Source: CAD feature listing. Evaluate the final solid. Frame: model axes, mm. A direction names the side the tool comes from. Give positions to 0.01 mm unless a question says otherwise; leave off trailing zeros. Order: outer loops, then holes, each group sorted by start corner. A loop starts at its lowest first (then second) coordinate and runs counter-clockwise, first axis right, second up. Notation, with made-up numbers: M 6.5,4 L 10.5,4 A16 ccw 10.5,16 Z; hole C 47.5,83 d2. An arc over 180 degrees is marked long. Answer as a JSON object with one key per item and string values. Group by question number.
1. Set-up query: faces 1 (the flat face through (15, 30, 15)), 2 (the flat face through (22.5, 55, 15)), 3 (the flat face through (65, 25, 15)), 4 (the cylindrical face through (3.7, 10.5, 13)). Return all of +Z, -Z, +X, -X, +Y, -Y with unobstructed straight access to the full face (end or side cutting, diameter ignored); none if empty.
2. Section query D-D (x = 25). Output: boundary loops of the cut face in (y, z), plus the area to 3 significant figures.
3. Section query B-B (y = 58). Output: boundary loops of the cut face in (x, z).
4. Material intervals for L1, parallel to Y at x = 6.25, z = 15; L2, parallel to Z at x = 2.5, y = 58; L3, parallel to X at y = 41.5, z = 13, sorted ascending. Write a range as [from, to].
5. Section query A-A (y = 12). Output: boundary loops of the cut face in (x, z), plus the area to 3 significant figures.
6. Pin query (flat end, axial travel): P1, Ø5, axis at x = 59, z = 26, coming from the +Y side; P2, Ø6, axis at x = 30.5, z = 17, coming from the -Y side; P3, Ø8, axis at y = 39.5, z = 7.5, coming from the +X side; P4, Ø7.5, axis at x = 13, z = 19, coming from the +Y side. Return the tip coordinate at first contact, or that it passes through.
7. Section query C-C (z = 15). Count the separate pieces of the cut face and the enclosed holes in it, plus the area to 3 significant figures.
8. Pull-direction query (X, two-part tool) for faces 5 (the flat face through (7.5, 15, 15)), 6 (the cylindrical face through (4, 68, 29)), 7 (the flat face through (15, 40, 15)), 8 (the flat face through (30, 50, 15)); classes: +X half, -X half, draft (parallel to the pull), parting line (faces both ways), or undercut.
from build123d import *

# Parameters (mm, degrees)
BOSS_EXTRUDE1_DEPTH = 30
SKETCH4_R           = 9
CUT_EXTRUDE2_DEPTH  = 25
SKETCH5_W           = 15
SKETCH5_H           = 30
CUT_EXTRUDE3_DEPTH  = 111.453610172
SKETCH6_R           = 2.5
CUT_EXTRUDE4_DEPTH  = 25
FILLET1_R           = 5
FILLET2_R           = 10


with BuildPart() as part:
    # Sketch1 → Boss-Extrude1 (new body)
    with BuildSketch(Plane.XY):
        Polygon((0, 0), (0, 70), (30, 70), (30, 30), (80, 30), (80, 0), align=None)
    extrude(amount=BOSS_EXTRUDE1_DEPTH)

    # Sketch4 → Cut-Extrude2 (cut)
    with BuildSketch(Plane(origin=(0, 0, 0), x_dir=(-1, 0, 0), z_dir=(0, -1, 0))):
        with Locations(Location((-65, -15, 0), (0, 0, 180))):
            Circle(SKETCH4_R)
    extrude(amount=-CUT_EXTRUDE2_DEPTH, mode=Mode.SUBTRACT)

    # Sketch5 → Cut-Extrude3 (cut, through all)
    with BuildSketch(Plane(origin=(0, 0, 0), x_dir=(-1, 0, 0), z_dir=(0, 0, -1))):
        with Locations((-15, 55)):
            Rectangle(SKETCH5_W, SKETCH5_H)
        with Locations((-15, 15)):
            Rectangle(SKETCH5_W, SKETCH5_H)
    extrude(amount=-CUT_EXTRUDE3_DEPTH, mode=Mode.SUBTRACT)

    # Sketch6 → Cut-Extrude4 (cut, symmetric)
    with BuildSketch(Plane.ZY.offset(-22.5)):
        with Locations(Location((15, 58, 0), (0, 0, 270))):
            Circle(SKETCH6_R)
        with Locations((15, 12)):
            Circle(SKETCH6_R)
    extrude(amount=CUT_EXTRUDE4_DEPTH, both=True, mode=Mode.SUBTRACT)

    # Fillet1
    fillet1_edges = [part.edges().sort_by_distance(p)[0] for p in [
        (26.25, 70, 30),
        (3.75, 70, 0),
        (3.75, 70, 30),
        (3.75, 0, 30),
        (26.25, 70, 0),
        (3.75, 0, 0),
    ]]
    fillet(fillet1_edges, radius=FILLET1_R)

    # Fillet2
    fillet2_edges = [part.edges().sort_by_distance(p)[0] for p in [
        (80, 15, 30),
        (80, 15, 0),
    ]]
    fillet(fillet2_edges, radius=FILLET2_R)


solid = part.part
Answer sheet:
{
 "1": {"face 1": "+Z, -Z, -Y", "face 2": "+Z, -Z, +Y", "face 3": "-Y", "face 4": "-X"},
 "2": {"outline": "M 0,0 L 65,0 A5 ccw 70,5 L 70,25 A5 ccw 65,30 L 0,30 Z; hole C 12,15 d5; hole C 58,15 d5", "area": "2,050 mm^2"},
 "3": {"outline": "M 0,0 L 7.5,0 L 7.5,12.5 L 0,12.5 Z; M 0,17.5 L 7.5,17.5 L 7.5,30 L 0,30 Z; M 22.5,0 L 30,0 L 30,12.5 L 22.5,12.5 Z; M 22.5,17.5 L 30,17.5 L 30,30 L 22.5,30 Z"},
 "4": {"L1": "[0, 9.5], [14.5, 55.5], [60.5, 70]", "L2": "[0, 12.5], [17.5, 30]", "L3": "[0, 7.5], [22.5, 30]"},
 "5": {"outline": "M 0,0 L 7.5,0 L 7.5,12.5 L 0,12.5 Z; M 0,17.5 L 7.5,17.5 L 7.5,30 L 0,30 Z; M 22.5,0 L 70,0 A10 ccw 80,10 L 80,20 A10 ccw 70,30 L 22.5,30 L 22.5,17.5 L 47.5,17.5 L 47.5,12.5 L 22.5,12.5 Z; hole C 65,15 d18", "area": "1,490 mm^2"},
 "6": {"P1": "y = 30", "P2": "y = 0", "P3": "x = 30", "P4": "y = 40"},
 "7": {"separate pieces": "4", "enclosed holes": "0", "area": "2,010 mm^2"},
 "8": {"face 5": "undercut", "face 6": "draft", "face 7": "undercut", "face 8": "+X half"}
}
